Read the model definition and answer for the solid it produces. Units are mm, in the model's axes. Face numbers are marked on the shaded views. A direction names the side the tool comes from. Give positions to 0.01 mm unless a question says otherwise; leave off trailing zeros. Loops run counter-clockwise (first coordinate to the right, second up) from the corner with the lowest first, then second, coordinate; pieces in that order, holes last. Notation, with made-up numbers: (-12, 47) -> (-1, 47) arc R21 cw to (-1, 53) -> close; hole circle Ø6 at (-25, 36.5). An arc over 180 degrees is marked (long way). Answer as CSV lines item,"result". Start each with the question number.
```python
from build123d import *

# Parameters (mm, degrees)
SKETCH_1_W                = 80
SKETCH_1_H                = 170
EXTRUDE_1_DEPTH           = 5
HOLE_WIZARD_1_D           = 10
HOLE_WIZARD_1_CBORE_D     = 12
HOLE_WIZARD_1_CBORE_DEPTH = 8
CUT_EXTRUDE_2_DEPTH       = 95.472218138
CUT_EXTRUDE_4_DEPTH       = 95.472218138
FILLET_1_R                = 5
HOLE_WIZARD_M6_1_D        = 5
HOLE_WIZARD_M6_1_DEPTH    = 17
HOLE_WIZARD_M6_1_TIP      = 1.502151548
HOLE_WIZARD_M4_1_D        = 3.3


with BuildPart() as part:
    # 草图1 → 凸台-拉伸1 (new, symmetric)
    with BuildSketch(Plane.XY):
        Rectangle(SKETCH_1_W, SKETCH_1_H)
    extrude(amount=EXTRUDE_1_DEPTH, both=True)

    # 孔1 (through all)
    with Locations(Plane(origin=(0, 0, 5), x_dir=(-1, 0, 0), z_dir=(0, 0, 1))):
        with Locations((0, 10)):
            CounterBoreHole(HOLE_WIZARD_1_D / 2, HOLE_WIZARD_1_CBORE_D / 2, HOLE_WIZARD_1_CBORE_DEPTH)

    # 草图6 → 切除-拉伸2 (cut, through all)
    with BuildSketch(Plane(origin=(0, 0, -5), x_dir=(-1, 0, 0), z_dir=(0, 0, -1))):
        with BuildLine():
            ThreePointArc((-14.125, -34.465217657), (7.311638024, -37.287404593), (24.465217657, -24.125))
            ThreePointArc((24.465217657, -24.125), (23.275635095, -19.685417438), (18.836052532, -20.875))
            ThreePointArc((18.836052532, -20.875), (5.629314231, -31.008886722), (-10.875, -28.836052532))
            ThreePointArc((-10.875, -28.836052532), (-15.314582562, -30.025635095), (-14.125, -34.465217657))
        make_face()
    extrude(amount=-CUT_EXTRUDE_2_DEPTH, mode=Mode.SUBTRACT)

    # 草图11 → 切除-拉伸4 (cut, through all)
    with BuildSketch(Plane(origin=(0, 0, -5), x_dir=(-1, 0, 0), z_dir=(0, 0, -1))):
        with BuildLine():
            Line((0, -46), (15, -46))
            Line((15, -46), (40, -21))
            Line((40, -21), (40, -85))
            Line((40, -85), (-40, -85))
            Line((-40, -85), (-40, 65))
            Line((-40, 65), (7.392754444, 25.232757226))
            ThreePointArc((7.392754444, 25.232757226), (-35.807675575, -6.283769392), (0, -46))
        make_face()
    extrude(amount=-CUT_EXTRUDE_4_DEPTH, mode=Mode.SUBTRACT)

    # 圆角1
    fillet_1_edges = [part.edges().sort_by_distance(p)[0] for p in [
        (-40, -21, 0),
        (-7.392754444, 25.232757226, 0),
        (-15, -46, 0),
    ]]
    fillet(fillet_1_edges, radius=FILLET_1_R)

    # M6 螺纹孔1
    with Locations(Plane(origin=(0, 85, 0), x_dir=(1, 0, 0), z_dir=(0, 1, 0))):
        with Locations((-28, 0), (28, 0)):
            Hole(HOLE_WIZARD_M6_1_D / 2, depth=HOLE_WIZARD_M6_1_DEPTH)
            with Locations((0, 0, -(HOLE_WIZARD_M6_1_DEPTH + HOLE_WIZARD_M6_1_TIP / 2))):  # 118° drill point
                Cone(0, HOLE_WIZARD_M6_1_D / 2, HOLE_WIZARD_M6_1_TIP, mode=Mode.SUBTRACT)

    # M4 螺纹孔1 (through all)
    with Locations(Plane(origin=(0, 0, -5), x_dir=(-1, 0, 0), z_dir=(0, 0, -1))):
        with Locations((20, 35), (20, 65), (20, 5)):
            Hole(HOLE_WIZARD_M4_1_D / 2)


solid = part.part
```
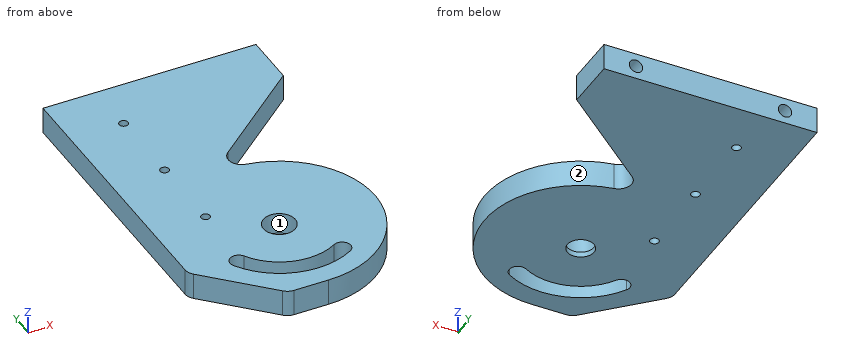
(1) Find the intervals of material crossed by line 1 along Z through (x, y) = (28, 74); line 2 along Y through (x, z) = (1, -3.25); line 3 along Y through (x, z) = (-20, 0.5), in increasing order. Write a range as from..to.
(2) Find section A-A on x = 12.5. Write down the section's boundary in (y, z).
(3) A tool of negligible diameter and unlimited length cuts with its end or side. For the marked faces 1 and 2, from which of +Z, -Z, +X, -X, +Y, -Y can it reach the whole face along a straight path? Write none if from no direction.
(4) Find section C-C on x = 33.5. Write down the section's boundary in (y, z), then the cut area to 3 significant figures.
(5) Each of these flat-tipped pins is pushed along its axis until it touches: P1, Ø7, axis at x = 0, y = -10, coming from the +Z side; P2, Ø1, axis at x = -19, z = 0, coming from the -Y side; P3, Ø9.5, axis at x = -0.5, y = -9.5, coming from the +Z side. Where does it stop, or does it pass through?
(6) Find section B-B on y = -36.5. Write down the section's boundary in (x, z).
(7) Find section D-D on y = 72. Write down the section's boundary in (x, z), then the cut area to 3 significant figures.
Answer block:
1,line 1,"z = -5..-2.5, 2.5..5"
1,line 2,"y = -45.99..-38.23, -31.73..-14.9, -5.1..85"
1,line 3,"y = -41..-29.95, -19.7..3.35, 6.65..33.35, 36.65..63.35, 66.65..85"
2,outline,"(-43.76, -5) -> (-35.33, -5) -> (-35.33, 5) -> (-43.76, 5) -> close; (-28.4, -5) -> (23.76, -5) -> (23.76, 5) -> (-28.4, 5) -> close; (41.92, -5) -> (85, -5) -> (85, 5) -> (41.92, 5) -> close"
3,face 1,"+Z"
3,face 2,"+Z, -Z, +X"
4,outline,"(-23.18, -5) -> (3.18, -5) -> (3.18, 5) -> (-23.18, 5) -> close; (59.55, -5) -> (85, -5) -> (85, 5) -> (59.55, 5) -> close"
4,area,"518 mm2"
5,P1,"passes through"
5,P2,"stops at y = -42.5"
5,P3,"stops at z = -3"
6,outline,"(-24.5, -5) -> (-9.79, -5) -> (-9.79, 5) -> (-24.5, 5) -> close; (9.79, -5) -> (24.37, -5) -> (24.37, 5) -> (9.79, 5) -> close"
7,outline,"(-40, -5) -> (40, -5) -> (40, 5) -> (-40, 5) -> close; hole circle Ø5 at (-28, 0); hole circle Ø5 at (28, 0)"
7,area,"761 mm2"
